from build123d import *

# Parameters (mm, degrees)
SKETCH_1_W                   = 50
SKETCH_1_H                   = 200
EXTRUDE_1_DEPTH              = 10
HOLE_WIZARD_M6_1_D           = 6.6
HOLE_WIZARD_M6_1_CBORE_D     = 11
HOLE_WIZARD_M6_1_CBORE_DEPTH = 8
HOLE_WIZARD_M6_1_2_D         = 5.2
HOLE_WIZARD_M6_1_2_DEPTH     = 15
HOLE_WIZARD_M6_1_2_TIP       = 1.562237609
HOLE_WIZARD_M6_2_D           = 5.2
HOLE_WIZARD_M6_2_CBORE_D     = 11
HOLE_WIZARD_M6_2_CBORE_DEPTH = 6.4
CHAMFER_1_SIZE               = 3


with BuildPart() as part:
    # 草图1 → 凸台-拉伸1 (new, symmetric)
    with BuildSketch(Plane(origin=(0, 0, 0), x_dir=(1, 0, 0), z_dir=(0, 1, 0))):
        Rectangle(SKETCH_1_W, SKETCH_1_H)
    extrude(amount=EXTRUDE_1_DEPTH, both=True)

    # Hole Wizard M6 _1 (through all)
    with Locations(Plane(origin=(0, 10, 0), x_dir=(1, 0, 0), z_dir=(0, 1, 0))):
        with Locations((0, 70), (0, -70), (0, 25), (0, -25)):
            CounterBoreHole(HOLE_WIZARD_M6_1_D / 2, HOLE_WIZARD_M6_1_CBORE_D / 2, HOLE_WIZARD_M6_1_CBORE_DEPTH)

    # Hole Wizard M6 _1 2
    with Locations(Plane(origin=(25, 0, 0), x_dir=(0, 0, -1), z_dir=(1, 0, 0))):
        with Locations((-85, 0), (0, 0), (85, 0)):
            Hole(HOLE_WIZARD_M6_1_2_D / 2, depth=HOLE_WIZARD_M6_1_2_DEPTH)
            with Locations((0, 0, -(HOLE_WIZARD_M6_1_2_DEPTH + HOLE_WIZARD_M6_1_2_TIP / 2))):  # 118° drill point
                Cone(0, HOLE_WIZARD_M6_1_2_D / 2, HOLE_WIZARD_M6_1_2_TIP, mode=Mode.SUBTRACT)

    # M6 六角凹头螺钉的柱形沉头孔2 (through all)
    with Locations(Plane(origin=(0, -10, 0), x_dir=(-1, 0, 0), z_dir=(0, -1, 0))):
        with Locations((0, 0)):
            CounterBoreHole(HOLE_WIZARD_M6_2_D / 2, HOLE_WIZARD_M6_2_CBORE_D / 2, HOLE_WIZARD_M6_2_CBORE_DEPTH)

    # 倒角1
    chamfer_1_edges = [part.edges().sort_by_distance(p)[0] for p in [
        (-25, 0, -100),
        (-25, 0, 100),
    ]]
    chamfer(chamfer_1_edges, length=CHAMFER_1_SIZE)


solid = part.part
Could you check a few things on this model? Use its own coordinates, in mm. A direction names the side the tool comes from. Give positions to 0.01 mm unless a question says otherwise; leave off trailing zeros. Write each loop counter-clockwise with the first axis right and the second up, starting at its lowest first coordinate (ties: lowest second). Pieces come first, ordered by that corner, then holes. Notation, with made-up numbers: (-36.5, 55) - (-14.5, 55) arc R22 ccw to (-14.5, 78) - close; hole circle Ø2 at (81.25, 72). An arc over 180 degrees is marked (long way). Use CSV: the item, a comma, the result in double quotes. Start each with the question number.
Item 1: I want a section at C-C, the plane x = 12.5. Please give me the cut outline in (y, z).
Item 2: If we mould it in two halves opening along Y, with no side actions, what happens to faces 5 (the face through (1, 0, 100)), 6 (the face through (0, 2, 29)), 7 (the face through (8.71, 0.14, -85.43))? For each: pulls with the +Y half, pulls with the -Y half, needs draft (parallel to the pull), parting line crosses it, or undercut.
Item 3: I'm going to push flat-ended pins straight in: pin 1 (9 mm diameter, centred on x = 0, z = 0, fed in from -Y); pin 2 (4 mm diameter, centred on x = 0, z = -25, fed in from +Y); pin 3 (10.5 mm diameter, centred on x = 0, z = 70, fed in from +Y); pin 4 (17.5 mm diameter, centred on x = 0, z = 70, fed in from -Y). Where does each tip first touch, or does it pass through?
Item 4: If I drill on line 1 along Z through (x, y) = (0, 5.75); line 2 along Z through (x, y) = (0, -4.75); line 3 along Y through (x, z) = (15, -85), over which ranges is the centre line in solid material (lowest first)?
Item 5: For faces 1 (the face through (17.395, 2.578, -0.338)), 2 (the face through (-0.338, 3.295, -2.578)), 3 (the face through (-4.05, 6.06, -28.72)), 4 (the face through (1.19, -6.84, 5.37)), which set-ups out of +Z, -Z, +X, -X, +Y, -Y let a thin tool reach every point of the face, with its end or its side?
Item 6: I want a section at B-B, the plane y = 4.5. Please give me the cut outline in (x, z), then the cut area to 3 significant figures.
Item 7: I want a section at A-A, the plane z = -70. Please give me the cut outline in (x, y).
Item 8: I want a section at D-D, the plane x = 0. Give the number of separate pieces and of enclosed holes in the cut face, then the cut area to 3 significant figures.
Findings:
1,outline,"(-10, -100) - (10, -100) - (10, 100) - (-10, 100) - close; hole circle Ø5.2 at (0, -85); hole circle Ø5.2 at (0, 0); hole circle Ø5.2 at (0, 85)"
2,face 5,"needs draft"
2,face 6,"pulls with the +Y half"
2,face 7,"undercut"
3,pin 1,"stops at y = -3.6"
3,pin 2,"passes through"
3,pin 3,"stops at y = 2"
3,pin 4,"stops at y = -10"
4,line 1,"z = -100 to -75.5, -64.5 to -30.5, -19.5 to -2.6, 2.6 to 19.5, 30.5 to 64.5, 75.5 to 100"
4,line 2,"z = -100 to -73.3, -66.7 to -28.3, -21.7 to -5.5, 5.5 to 21.7, 28.3 to 66.7, 73.3 to 100"
4,line 3,"y = -10 to -2.6, 2.6 to 10"
5,face 1,"+X"
5,face 2,"+Y, -Y"
5,face 3,"+Y"
5,face 4,"-Y"
6,outline,"(-25, -97) - (-22, -100) - (25, -100) - (25, 100) - (-22, 100) - (-25, 97) - close; hole circle Ø11 at (0, -70); hole circle Ø11 at (0, -25); hole circle Ø11 at (0, 25); hole circle Ø11 at (0, 70); hole circle Ø5.2 at (0, 0)"
6,area,"9,590 mm2"
7,outline,"(-25, -10) - (-3.3, -10) - (-3.3, 2) - (-5.5, 2) - (-5.5, 10) - (-25, 10) - close; (3.3, -10) - (25, -10) - (25, 10) - (5.5, 10) - (5.5, 2) - (3.3, 2) - close"
8,separate pieces,"6"
8,enclosed holes,"0"
8,area,"3,190 mm2"
